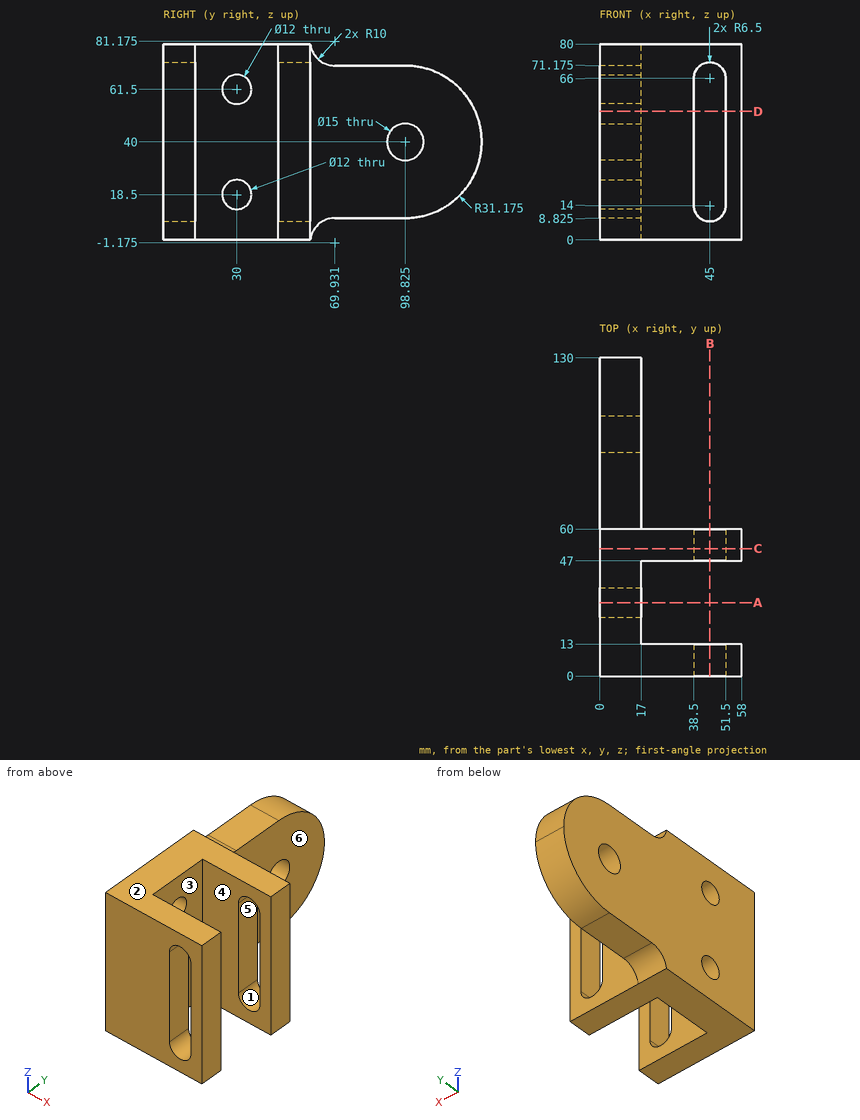
Print and shaded views of the part. All mm, measured from the part's lowest x, y and z. A direction names the side the tool comes from. Coordinates: 2 decimals unless noted, no trailing zeros. Loops run counter-clockwise (first coordinate to the right, second up) from the corner with the lowest first, then second, coordinate; pieces in that order, holes last. Notation, with made-up numbers: M 7.25,-26 L 46.25,-26 A23 cw 46.25,-12 Z; hole C 29,47.25 d1. An arc over 180 degrees is marked long. Use a Markdown table: item, result. Add a question column.
Q1. Cut at D-D (z = 52.5). Write the cut outline in (x, y), and give its area (3 significant figures).
Q2. Which spindle directions (+Z, -Z, +X, -X, +Y, -Y) get a long thin tool onto all of the face, cutting with end or side? Do the marked faces 4, 5 and 6. Say none if no direction does.
Q3. Probe L1, parallel to Y at x = 29.5, z = 21.5; L2, parallel to X at y = 52.5, z = 38; L3, parallel to X at y = 90.5, z = 68.5. List the from-to ranges inside material, lowest first.
Q4. Pin check, flat tips, straight feed: P1, Ø18.5, axis at x = 6, y = 83.5, coming from the +Z side (1 decimal); P2, Ø4, axis at y = 4.5, z = 31, coming from the -X side; P3, Ø12.5, axis at x = 36, z = 24, coming from the +Y side; P4, Ø18.5, axis at x = 9.5, y = 87.5, coming from the -Z side (1 decimal). Stop position of each tip, or through.
Q5. Cut at B-B (x = 45). Write the cut outline in (y, z), and give its area (3 significant figures).
Q6. Mould opens along Z. For the marked faces 1, 2 and 3 say: +Z half, -Z half, draft (parallel to the pull), parting line (faces both ways), or undercut.
Q7. Cut at A-A (y = 30). Write the cut outline in (x, z).
Q8. Cut at C-C (y = 52). Write the cut outline in (x, z).
Worked out:
| question | item | result |
|---|---|---|
| 1 | outline | M 0,0 L 38.5,0 L 38.5,13 L 17,13 L 17,47 L 38.5,47 L 38.5,60 L 17,60 L 17,127.38 L 0,127.38 Z; M 51.5,0 L 58,0 L 58,13 L 51.5,13 Z; M 51.5,47 L 58,47 L 58,60 L 51.5,60 Z |
| 1 | area | 2,890 mm2 |
| 2 | face 4 | +Z, -Z, +X |
| 2 | face 5 | +Y, -Y |
| 2 | face 6 | +Z, -Z, +X, +Y |
| 3 | L1 | y = 0 to 13, 47 to 60 |
| 3 | L2 | x = 0 to 38.5, 51.5 to 58 |
| 3 | L3 | x = 0 to 17 |
| 4 | P1 | stops at z = 71.2 |
| 4 | P2 | stops at x = 0 |
| 4 | P3 | stops at y = 60 |
| 4 | P4 | stops at z = 8.8 |
| 5 | outline | M 0,0 L 13,0 L 13,7.5 L 0,7.5 Z; M 0,72.5 L 13,72.5 L 13,80 L 0,80 Z; M 47,0 L 60,0 L 60,7.5 L 47,7.5 Z; M 47,72.5 L 60,72.5 L 60,80 L 47,80 Z |
| 5 | area | 390 mm2 |
| 6 | face 1 | undercut |
| 6 | face 2 | +Z half |
| 6 | face 3 | draft |
| 7 | outline | M 0,0 L 17,0 L 17,12.5 L 0,12.5 Z; M 0,24.5 L 17,24.5 L 17,55.5 L 0,55.5 Z; M 0,67.5 L 17,67.5 L 17,80 L 0,80 Z |
| 8 | outline | M 0,0 L 58,0 L 58,80 L 0,80 Z; hole M 38.5,14 A6.5 ccw 51.5,14 L 51.5,66 A6.5 ccw 38.5,66 Z |
